Study the drawing (mm; zero at the part's minimum x, y, z) and answer. A direction names the side the tool comes from. Give positions to 0.01 mm unless a question says otherwise; leave off trailing zeros. Loops run counter-clockwise (first coordinate to the right, second up) from the corner with the lowest first, then second, coordinate; pieces in that order, holes last. Notation, with made-up numbers: (14, 45) - (19, 45) arc R24 cw to (19, 62) - close; hole circle Ø1 at (76.5, 31). An arc over 180 degrees is marked (long way). Write item = value, one per line. Start each with the question number.
1) The mould has two halves that part along Y. Classify the marked faces 1, 2, 3 and 4: +Y half, -Y half, draft (parallel to the pull), parting line (faces both ways), or undercut.
2) Flat-ended cylindrical pins translate along their axes: P1, Ø1, axis at x = 1, z = 3, coming from the -Y side; P2, Ø0.6, axis at y = 26, z = 3.5, coming from the +X side; P3, Ø1, axis at x = 1.5, z = 5, coming from the +Y side; P4, Ø6, axis at x = 11.5, y = 13.5, coming from the -Z side. Find the tip coordinate at first contact, or state that the pin passes through.
3) The part is cut by section A-A on x = 14. Write down the section's boundary in (y, z).
4) Which of the six approach directions +Z, -Z, +X, -X, +Y, -Y give full straight-line access (tool end or side, diameter ignored) to the marked faces 5, 6 and 7?
5) Consider probe 1 along Y at (x, z) = (12.5, 1); probe 2 along X at (y, z) = (11, 4.25); probe 3 along Y at (x, z) = (1.75, 2) (1 decimal). Determine where each line is inside the solid, lowest interval first.
6) The part is cut by section B-B on z = 1.5. Write down the section's boundary in (x, y).
7) The part is cut by section C-C on y = 12.25. Write down the section's boundary in (x, z).
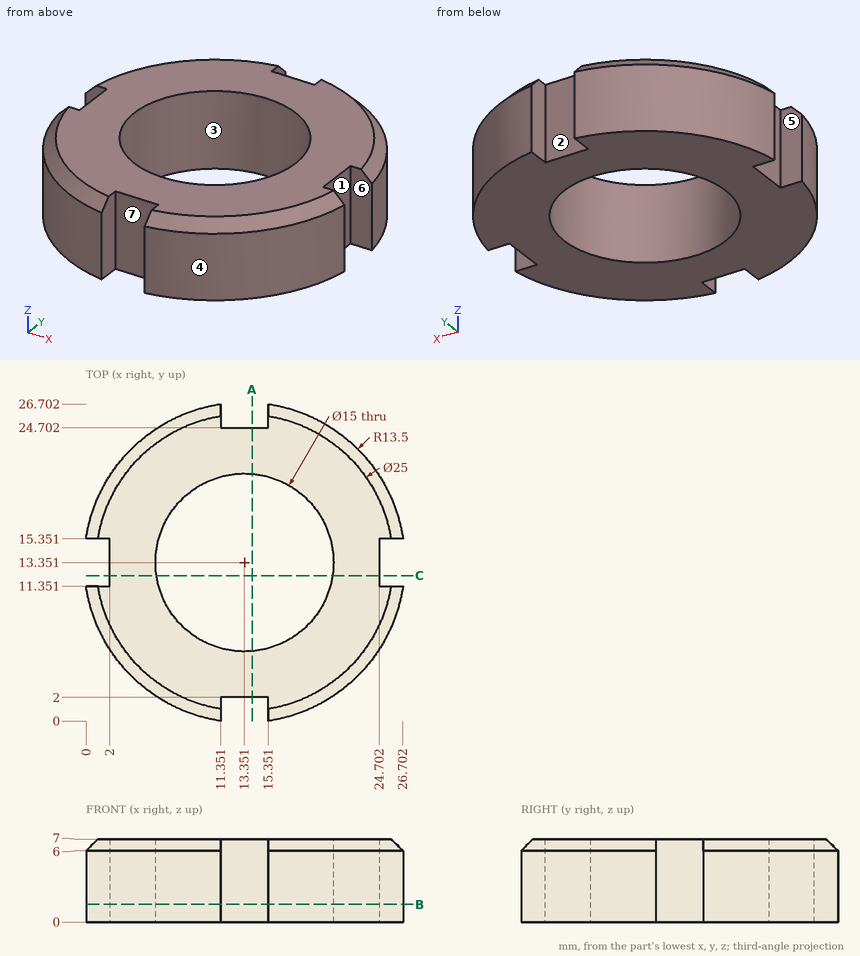
Answer below:
q1.face_1 = undercut
q1.face_2 = +Y half
q1.face_3 = undercut
q1.face_4 = -Y half
q2.P1 = 6.89
q2.P2 = 18.81
q2.P3 = 20.66
q2.P4 = through
q3.outline = (2, 0) - (5.88, 0) - (5.88, 7) - (2, 7) - close; (20.82, 0) - (24.7, 0) - (24.7, 7) - (20.82, 7) - close
q4.face_5 = +Z, -Z, -X
q4.face_6 = +Z, -Z, +X
q4.face_7 = +Z, -Z, -Y
q5.probe_1 = 2 to 5.9, 20.8 to 24.7
q5.probe_2 = 0.06 to 6.23, 20.47 to 26.64
q5.probe_3 = 6.4 to 11.4, 15.4 to 20.3
q6.outline = (0, 11.35) arc R13.5 ccw to (11.35, 0) - (11.35, 2) - (15.35, 2) - (15.35, 0) arc R13.5 ccw to (26.7, 11.35) - (24.7, 11.35) - (24.7, 15.35) - (26.7, 15.35) arc R13.5 ccw to (15.35, 26.7) - (15.35, 24.7) - (11.35, 24.7) - (11.35, 26.7) arc R13.5 ccw to (0, 15.35) - (2, 15.35) - (2, 11.35) - close; hole circle Ø15 at (13.35, 13.35)
q7.outline = (2, 0) - (5.93, 0) - (5.93, 7) - (2, 7) - close; (20.77, 0) - (24.7, 0) - (24.7, 7) - (20.77, 7) - close
